Verification items for the finished model (mm, model axes). Coordinates: 2 decimals unless noted, no trailing zeros. Order: outer loops, then holes, each group sorted by start corner. A loop starts at its lowest first (then second) coordinate and runs counter-clockwise, first axis right, second up.
Q1. Cross-section at B-B, the plane y = 0. Record the boundary of the cut face in (x, z).
Q2. Cross-section at A-A, the plane x = 1.25. Record the boundary of the cut face in (y, z), and give its area (3 significant figures).
Q3. Cross-section at C-C, the plane z = -0.35. Record the boundary of the cut face in (x, y).
Q4. Thickness scan on line 1 (Y direction, x = -10.75, z = 0.15); line 2 (X direction, y = -0.15, z = 0.15); line 3 (X direction, y = 0.4, z = 0.4). Record the ranges inside material, lowest first.
from build123d import *

# Parameters (mm, degrees)
SKETCH1_R           = 0.55
THIGH1_LENGTH_DEPTH = 0.5


with BuildPart() as part:
    # Sketch1 → Thigh1 length (new, symmetric)
    with BuildSketch(Plane.XY):
        with BuildLine():
            Line((-10.75, 1), (10.75, 1))
            ThreePointArc((10.75, 1), (11.75, 0), (10.75, -1))
            Line((10.75, -1), (-10.75, -1))
            ThreePointArc((-10.75, -1), (-11.75, 0), (-10.75, 1))
        make_face()
        with Locations((-10.75, 0)):
            Circle(SKETCH1_R, mode=Mode.SUBTRACT)
        with Locations((10.75, 0)):
            Circle(SKETCH1_R, mode=Mode.SUBTRACT)
        with Locations((1.25, 0)):
            Circle(SKETCH1_R, mode=Mode.SUBTRACT)
    extrude(amount=THIGH1_LENGTH_DEPTH, both=True)


solid = part.part
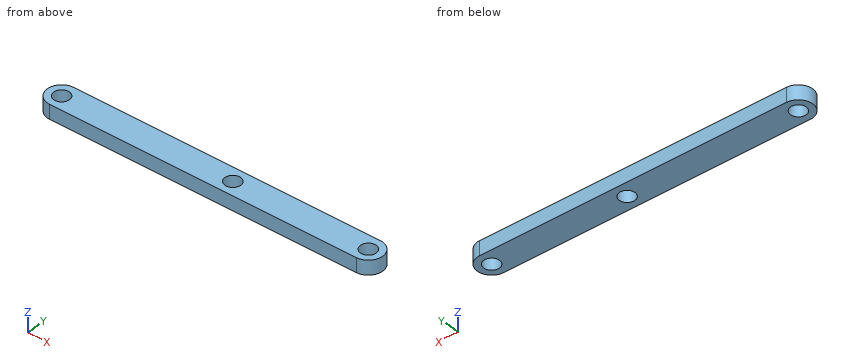
Check values:
1. outline: (-11.75, -0.5) - (-11.3, -0.5) - (-11.3, 0.5) - (-11.75, 0.5) - close; (-10.2, -0.5) - (0.7, -0.5) - (0.7, 0.5) - (-10.2, 0.5) - close; (1.8, -0.5) - (10.2, -0.5) - (10.2, 0.5) - (1.8, 0.5) - close; (11.3, -0.5) - (11.75, -0.5) - (11.75, 0.5) - (11.3, 0.5) - close
2. outline: (-1, -0.5) - (-0.55, -0.5) - (-0.55, 0.5) - (-1, 0.5) - close; (0.55, -0.5) - (1, -0.5) - (1, 0.5) - (0.55, 0.5) - close
2. area: 0.900 mm2
3. outline: (-10.75, -1) - (10.75, -1) arc R1 ccw to (10.75, 1) - (-10.75, 1) arc R1 ccw to start; hole circle Ø1.1 at (-10.75, 0); hole circle Ø1.1 at (1.25, 0); hole circle Ø1.1 at (10.75, 0)
4. line 1: y = -1 to -0.55, 0.55 to 1
4. line 2: x = -11.74 to -11.28, -10.22 to 0.72, 1.78 to 10.22, 11.28 to 11.74
4. line 3: x = -11.67 to -11.13, -10.37 to 0.87, 1.63 to 10.37, 11.13 to 11.67
